Here's how the part is built. I have some questions about the finished solid (model axes, mm). A direction names the side the tool comes from. Coordinates: 2 decimals unless noted, no trailing zeros. Order: outer loops, then holes, each group sorted by start corner. A loop starts at its lowest first (then second) coordinate and runs counter-clockwise, first axis right, second up. Notation, with made-up numbers: (5.25, 51.25) - (18.25, 51.25) arc R33 ccw to (18.25, 90.25) - close; hole circle Ø8 at (88.5, 37.25). An arc over 180 degrees is marked (long way). Use one line per item in the form item = value. Start each with the question number.
from build123d import *

# Parameters (mm, degrees)
HEX_HEAD_DEPTH     = 5
SHANK_PROFILE_12_R = 6
SHANK_12_DEPTH     = 27


with BuildPart() as part:
    # Hex Head Profile 20AF → Hex Head (new body)
    with BuildSketch(Plane(origin=(0, 0, 0), x_dir=(0, 0, -1), z_dir=(1, 0, 0))):
        Polygon((11.547005384, 0), (5.773502692, 10), (-5.773502692, 10), (-11.547005384, 0), (-5.773502692, -10), (5.773502692, -10), align=None)
    extrude(amount=HEX_HEAD_DEPTH)

    # Shank Profile Ø12 → Shank Ø12 (add)
    with BuildSketch(Plane.ZY):
        Circle(SHANK_PROFILE_12_R)
    extrude(amount=SHANK_12_DEPTH)

    # Head Chamfer Profile → Head Chamfer (revolve, cut)
    with BuildSketch(Plane(origin=(0, 0, 0), x_dir=(1, 0, 0), z_dir=(0, 1, 0)), mode=Mode.PRIVATE) as head_chamfer_sk:
        Polygon((2.5, 11.547005384), (5, 9.547005384), (5, 11.547005384), align=None)
    revolve(head_chamfer_sk.sketch.rotate(Axis((0, 0, 0), (1, 0, 0)), 180), axis=Axis((0, 0, 0), (1, 0, 0)), mode=Mode.SUBTRACT)


solid = part.part
1) Suppose I cut it at C-C, the plane x = -11.5. List the corners of the cut face in (y, z) for me, then the cut area to 3 significant figures.
2) Suppose I cut it at B-B, the plane x = 0.5. List the corners of the cut face in (y, z) for me, then the cut area to 3 significant figures.
3) I need wall thicknesses on probe 1 along X at (y, z) = (4.5, -6.25); probe 2 along X at (y, z) = (8, -6); probe 3 along Y at (x, z) = (-3, -3). Which ranges of each line are inside material? Lowest first, please. Write a range as [from, to].
4) For pin 1 (4 mm diameter, centred on y = -8, z = -3.5, fed in from -X); pin 2 (5 mm diameter, centred on y = 7, z = 7, fed in from +X); pin 3 (12 mm diameter, centred on x = 0.5, y = -6.5, fed in from +Z); pin 4 (5 mm diameter, centred on x = -19, y = 5, fed in from -Z), each with a flat end and sliding along its axis, tell me the tip position at first contact or that it passes through.
5) Which directions (+Z, -Z, +X, -X, +Y, -Y) give clear straight access to the entire face, cutting with the end or side of a thin tool? Please do faces 1 (the flat face through (1.69, -4.93, 8.7)), 2 (the cylindrical face through (-13, 0, -6)).
6) Suppose I cut it at A-A, the plane z = 0. List the corners of the cut face in (x, y) for me.
From the geometry:
q1.outline = circle Ø12 at (0, 0)
q1.area = 113 mm2
q2.outline = (-10, -5.77) - (0, -11.55) - (10, -5.77) - (10, 5.77) - (0, 11.55) - (-10, 5.77) - close
q2.area = 346 mm2
q3.probe_1 = [0, 5]
q3.probe_2 = [0, 4.43]
q3.probe_3 = [-5.2, 5.2]
q4.pin_1 = 0
q4.pin_2 = 5
q4.pin_3 = 11.26
q4.pin_4 = -5.45
q5.face_1 = +Z, +X, -X, -Y
q5.face_2 = -X
q6.outline = (-27, -6) - (0, -6) - (0, -10) - (4.43, -10) - (5, -9.55) - (5, 9.55) - (4.43, 10) - (0, 10) - (0, 6) - (-27, 6) - close
